from build123d import *

# Parameters (mm, degrees)
SKETCH_1_W              = 1172
SKETCH_1_H              = 36
EXTRUDE_1_DEPTH         = 4
CHAMFER_1_SIZE          = 5
HOLE_WIZARD_10_0_10_1_D = 10
PATTERN_LINEAR_1_COUNT  = 15
PATTERN_LINEAR_1_PITCH  = 80


with BuildPart() as part:
    # 草图1 → 凸台-拉伸1 (new body)
    with BuildSketch(Plane(origin=(0, 0, 0), x_dir=(1, 0, 0), z_dir=(0, 1, 0))):
        with Locations((-586, -18)):
            Rectangle(SKETCH_1_W, SKETCH_1_H)
    extrude(amount=EXTRUDE_1_DEPTH)

    # 倒角1
    chamfer_1_edges = [part.edges().sort_by_distance(p)[0] for p in [
        (-1172, 2, 0),
        (0, 2, 0),
    ]]
    chamfer(chamfer_1_edges, length=CHAMFER_1_SIZE)

    # Ø10.0 (10) 直径孔1 (through all)
    with Locations(Plane(origin=(0, 4, 0), x_dir=(-1, 0, 0), z_dir=(0, 1, 0))):
        with Locations((1151, 21)):
            hole_wizard_10_0_10_1 = Hole(HOLE_WIZARD_10_0_10_1_D / 2)

    # 阵列(线性)1: Ø10.0 (10) 直径孔1 ×15
    with Locations(*[(i * PATTERN_LINEAR_1_PITCH, 0, 0) for i in range(1, PATTERN_LINEAR_1_COUNT)]):
        add(hole_wizard_10_0_10_1, mode=Mode.SUBTRACT)


solid = part.part
Build history of the part. All positions in model axes, mm. Coordinates: 2 decimals unless noted, no trailing zeros. Write item = value, one per line. Start each with the question number.
1) Wall check: line 1 along Z through (x, y) = (-31, 3); line 2 along X through (y, z) = (1, 2). Give the ranges that are in metal, low to high. Write a range as from..to.
2) Saw through at A-A on y = 1.8. Count the separate pieces of the cut face and the enclosed holes in it, then the cut area to 3 significant figures.
3) Flat gauge pin, fed straight in: pin 1 Ø6 at (x, z) = (-431, 21) entering from -Y. Where does the tip first touch, or does it go through?
From the geometry:
q1.line_1 = 0..16, 26..36
q1.line_2 = -1169..-3
q2.separate_pieces = 1
q2.enclosed_holes = 15
q2.area = 41,000 mm^2
q3.pin_1 = through
